CAD build for the part. Positions are in the model's coordinates, mm. Face numbers are marked on the shaded views. Give positions to 0.01 mm unless a question says otherwise; leave off trailing zeros. Order: outer loops, then holes, each group sorted by start corner. A loop starts at its lowest first (then second) coordinate and runs counter-clockwise, first axis right, second up.
Item 1: Band-saw the part on B-B on y = -266. Give the cut face in (x, z).
Item 2: Band-saw the part on A-A on z = 23.5. Give the cut face in (x, y).
Item 3: Two-plate mould, pull along Y, no slides. Class the marked faces 1, 2, 3 and 4: released by +Y, released by -Y, zero draft, split by the parting line, or undercut.
Item 4: Wall check: L1, parallel to Y at x = -123, z = 19; L2, parallel to X at y = -176, z = 12. Give the ranges that are in metal, low to high.
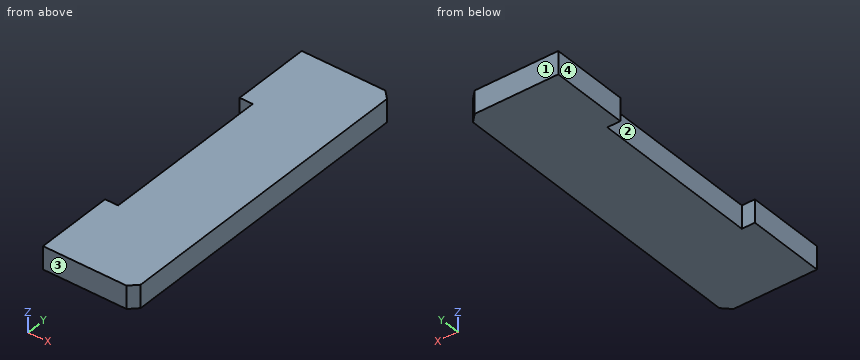
```python
from build123d import *

# Parameters (mm, degrees)
EXTRUDE_1_DEPTH = 35
CHAMFER_1_SIZE  = 12


with BuildPart() as part:
    # 草图1 → 凸台-拉伸1 (new body)
    with BuildSketch(Plane.XY):
        Polygon((-140, 0), (0, 0), (0, -500), (-140, -500), (-140, -380), (-120, -380), (-120, -120), (-140, -120), align=None)
    extrude(amount=EXTRUDE_1_DEPTH)

    # 倒角1
    chamfer_1_edges = [part.edges().sort_by_distance(p)[0] for p in [
        (0, -500, 17.5),
        (0, 0, 17.5),
    ]]
    chamfer(chamfer_1_edges, length=CHAMFER_1_SIZE)


solid = part.part
```
The answers:
1. outline: (-120, 0) - (0, 0) - (0, 35) - (-120, 35) - close
2. outline: (-140, -500) - (-12, -500) - (0, -488) - (0, -12) - (-12, 0) - (-140, 0) - (-140, -120) - (-120, -120) - (-120, -380) - (-140, -380) - close
3. face 1: released by +Y
3. face 2: undercut
3. face 3: released by -Y
3. face 4: zero draft
4. L1: y = -500 to -380, -120 to 0
4. L2: x = -120 to 0
